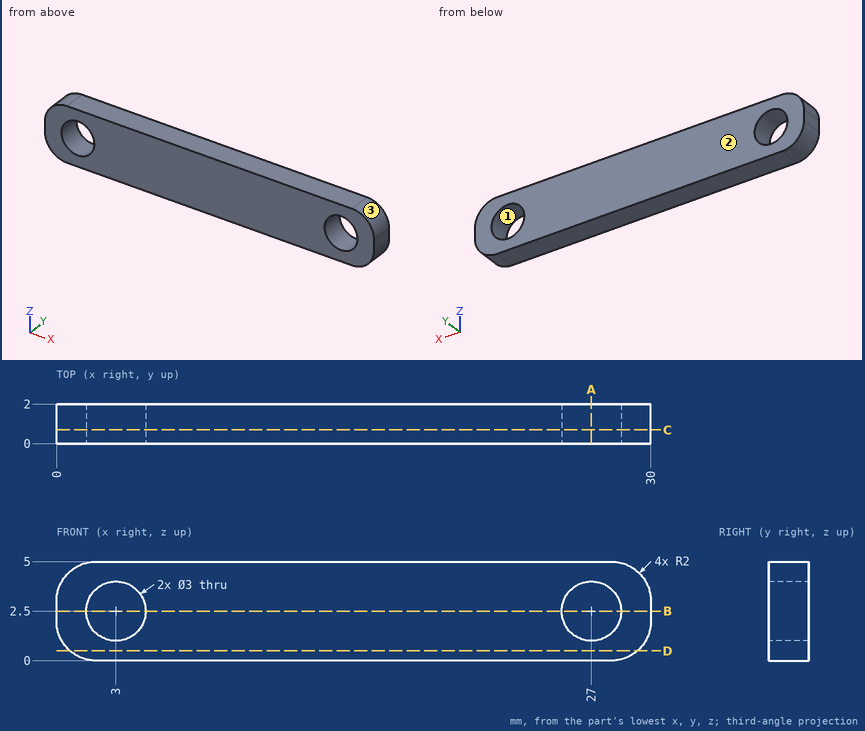
Study the drawing (mm; zero at the part's minimum x, y, z) and answer. Give positions to 0.01 mm unless a question says otherwise; leave off trailing zeros. Loops run counter-clockwise (first coordinate to the right, second up) from the corner with the lowest first, then second, coordinate; pieces in that order, holes last. Notation, with made-up numbers: (81, 66.25) - (110, 66.25) arc R30 ccw to (110, 98.25) - close; hole circle Ø4 at (33.25, 87). An arc over 180 degrees is marked (long way). Answer in a Markdown table with one row per item. Add a question column.
Q1. The part is cut by section D-D (z = 0.5). Determine the outline of the cut face in (x, y).
Q2. The part is cut by section C-C (y = 0.7). Determine the outline of the cut face in (x, z).
Q3. The part is cut by section B-B (z = 2.5). Determine the outline of the cut face in (x, y), and give its area (3 significant figures).
Q4. Consider line 1 along X through (y, z) = (0.75, 2.5); line 2 along X through (y, z) = (1.3, 3.3); line 3 along Z through (x, y) = (4, 1.5). Determine where each line is inside the solid, lowest interval first.
Q5. The part is cut by section A-A (x = 27). Determine the outline of the cut face in (y, z).
Q6. Determine the mould class of the marked faces 1, 2 and 3 for opening direction Z: released by +Z, released by -Z, zero draft, split by the parting line, or undercut.
Solution:
| question | item | result |
|---|---|---|
| 1 | outline | (0.68, 0) - (29.32, 0) - (29.32, 2) - (0.68, 2) - close |
| 2 | outline | (0, 2) arc R2 ccw to (2, 0) - (28, 0) arc R2 ccw to (30, 2) - (30, 3) arc R2 ccw to (28, 5) - (2, 5) arc R2 ccw to (0, 3) - close; hole circle Ø3 at (3, 2.5); hole circle Ø3 at (27, 2.5) |
| 3 | outline | (0, 0) - (1.5, 0) - (1.5, 2) - (0, 2) - close; (4.5, 0) - (25.5, 0) - (25.5, 2) - (4.5, 2) - close; (28.5, 0) - (30, 0) - (30, 2) - (28.5, 2) - close |
| 3 | area | 48.0 mm² |
| 4 | line 1 | x = 0 to 1.5, 4.5 to 25.5, 28.5 to 30 |
| 4 | line 2 | x = 0.02 to 1.73, 4.27 to 25.73, 28.27 to 29.98 |
| 4 | line 3 | z = 0 to 1.38, 3.62 to 5 |
| 5 | outline | (0, 0) - (2, 0) - (2, 1) - (0, 1) - close; (0, 4) - (2, 4) - (2, 5) - (0, 5) - close |
| 6 | face 1 | undercut |
| 6 | face 2 | zero draft |
| 6 | face 3 | released by +Z |
